Check sheet for the modelled part. Datum: model origin and axes. Units: mm. Round coordinates to 2 decimals unless told otherwise and drop trailing zeros. Order: outer loops, then holes, each group sorted by start corner. A loop starts at its lowest first (then second) coordinate and runs counter-clockwise, first axis right, second up.
```python
from build123d import *

# Parameters (mm, degrees)
EXTRUDE_1_DEPTH = 705


with BuildPart() as part:
    # 草图1 → 凸台-拉伸1 (new, symmetric)
    with BuildSketch(Plane.XY):
        with BuildLine():
            Line((-4.556913863, 4.138102128), (-2.645672962, 1.79891143))
            Line((-2.645672962, 1.79891143), (-5, 1.79891143))
            Line((-5, 1.79891143), (-5, 1.29891143))
            Line((-5, 1.29891143), (1.591473901, 1.29891143))
            Line((1.591473901, 1.29891143), (5, 1.29891143))
            Line((5, 1.29891143), (5, 1.79891143))
            Line((5, 1.79891143), (2.645672962, 1.79891143))
            Line((2.645672962, 1.79891143), (4.556913863, 4.138102128))
            ThreePointArc((4.556913863, 4.138102128), (4.780792009, 4.829714088), (4.47713902, 5.490201325))
            ThreePointArc((4.47713902, 5.490201325), (0, 7.29891143), (-4.47713902, 5.490201325))
            ThreePointArc((-4.47713902, 5.490201325), (-4.780792009, 4.829714088), (-4.556913863, 4.138102128))
        make_face()
        with BuildLine():
            Line((-2, 1.79891143), (2, 1.79891143))
            Line((2, 1.79891143), (4.169720942, 4.454458955))
            ThreePointArc((4.169720942, 4.454458955), (4.281660015, 4.800264935), (4.12983352, 5.130508554))
            ThreePointArc((4.12983352, 5.130508554), (0, 6.79891143), (-4.12983352, 5.130508554))
            ThreePointArc((-4.12983352, 5.130508554), (-4.281660015, 4.800264935), (-4.169720942, 4.454458955))
            Line((-4.169720942, 4.454458955), (-2, 1.79891143))
        make_face(mode=Mode.SUBTRACT)
    extrude(amount=EXTRUDE_1_DEPTH, both=True)


solid = part.part
```
Item 1: Go/stop test with flat-tipped pins: P1, Ø1.5, axis at y = 4.5, z = -169, coming from the -X side; P2, Ø1.2, axis at x = 4, z = 298, coming from the +Y side; P3, Ø3, axis at x = -1, z = 108.5, coming from the +Y side; P4, Ø1.5, axis at x = 2, z = 346.5, coming from the +Y side. Record where each tip stops, or that it passes through.
Answer:
P1: stops at x = -4.78
P2: stops at y = 6.33
P3: stops at y = 7.3
P4: stops at y = 7.18
Item 2: Scan lines: line 1 along X through (y, z) = (2.1, -390.5); line 2 along Y through (x, z) = (-0.75, 337.5); line 3 along Y through (x, z) = (-3.5, 324.5). Record each from-to range of solid material in increasing order.
Answer:
line 1: x = -2.89 to -2.25, 2.25 to 2.89
line 2: y = 1.3 to 1.8, 6.75 to 7.26
line 3: y = 1.3 to 1.8, 2.84 to 3.63, 5.66 to 6.27
Item 3: Sectioned sample at B-B (y = 2.75). Record the cut outline in (x, z).
Answer:
outline: (-3.42, -705) - (-2.78, -705) - (-2.78, 705) - (-3.42, 705) - close; (2.78, -705) - (3.42, -705) - (3.42, 705) - (2.78, 705) - close
Item 4: Sectioned sample at A-A (z = -544). Record the cut outline in (x, y).
Answer:
outline: (-5, 1.3) - (5, 1.3) - (5, 1.8) - (2.65, 1.8) - (4.56, 4.14) arc R1 ccw to (4.48, 5.49) arc R6.45 ccw to (-4.48, 5.49) arc R1 ccw to (-4.56, 4.14) - (-2.65, 1.8) - (-5, 1.8) - close; hole (-4.17, 4.45) - (-2, 1.8) - (2, 1.8) - (4.17, 4.45) arc R0.5 ccw to (4.13, 5.13) arc R5.95 ccw to (-4.13, 5.13) arc R0.5 ccw to start
